```python
from build123d import *

# Parameters (mm, degrees)
COLD_FORMED_SQUARE_HOLLOW_SECTION_GB_T_6_DEPTH = 300


with BuildPart() as part:
    # Sketch1 → Cold-formed square hollow section GB/T 6728-2002 50 X 50 X 4(1) (new body)
    with BuildSketch(Plane.YZ.offset(-88.434077868)):
        with BuildLine():
            Line((-17, -25), (17, -25))
            ThreePointArc((17, -25), (22.656854249, -22.656854249), (25, -17))
            Line((25, -17), (25, 17))
            ThreePointArc((25, 17), (22.656854249, 22.656854249), (17, 25))
            Line((17, 25), (-17, 25))
            ThreePointArc((-17, 25), (-22.656854249, 22.656854249), (-25, 17))
            Line((-25, 17), (-25, -17))
            ThreePointArc((-25, -17), (-22.656854249, -22.656854249), (-17, -25))
        make_face()
        with BuildLine():
            Line((-17, -20), (17, -20))
            ThreePointArc((17, -20), (19.121320344, -19.121320344), (20, -17))
            Line((20, -17), (20, 17))
            ThreePointArc((20, 17), (19.121320344, 19.121320344), (17, 20))
            Line((17, 20), (-17, 20))
            ThreePointArc((-17, 20), (-19.121320344, 19.121320344), (-20, 17))
            Line((-20, 17), (-20, -17))
            ThreePointArc((-20, -17), (-19.121320344, -19.121320344), (-17, -20))
        make_face(mode=Mode.SUBTRACT)
    extrude(amount=COLD_FORMED_SQUARE_HOLLOW_SECTION_GB_T_6_DEPTH)


solid = part.part
```
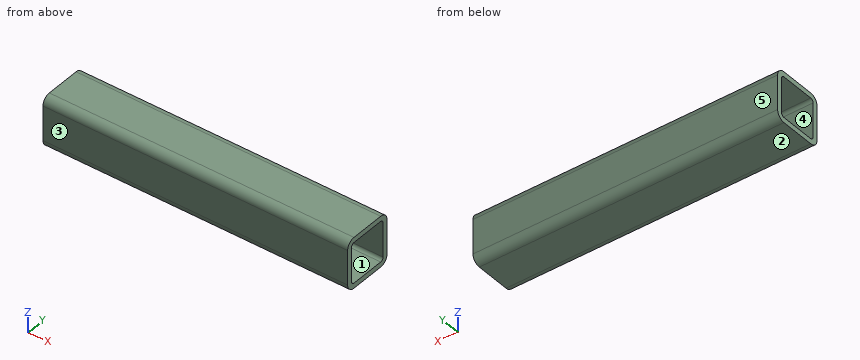
Read the model definition and answer for the solid it produces. Units are mm, in the model's axes. Face numbers are marked on the shaded views. A direction names the side the tool comes from. Coordinates: 2 decimals unless noted, no trailing zeros. Write each loop counter-clockwise with the first axis right and the second up, starting at its lowest first coordinate (ties: lowest second). Pieces come first, ordered by that corner, then holes. Notation, with made-up numbers: (49.5, 89) - (85.5, 89) arc R27 ccw to (85.5, 109) - close; hole circle Ø10 at (10, -11.75). An arc over 180 degrees is marked (long way). Answer as a JSON object with one key per item and string values. Group by question number.
1. A cutting plane is placed at A-A (z = -9). Determine the outline of the cut face in (x, y).
2. Consider L1, parallel to Y at x = 39.5, z = 11; L2, parallel to Y at x = 61, z = 18. Determine where each line is inside the solid, lowest interval first. Write a range as [from, to].
3. A cutting plane is placed at D-D (y = 22.5). Determine the outline of the cut face in (x, z).
4. The mould has two halves that part along Y. Classify the marked faces 1, 2 and 3: +Y half, -Y half, draft (parallel to the pull), parting line (faces both ways), or undercut.
5. Each of these flat-tipped pins is pushed along its axis until it touches: P1, Ø4, axis at x = 171, y = 19.5, coming from the +Z side; P2, Ø4, axis at x = -13.5, y = 20, coming from the +Z side. Where does it stop, or does it pass through?
6. Which of the six approach directions +Z, -Z, +X, -X, +Y, -Y give full straight-line access (tool end or side, diameter ignored) to the marked faces 4 and 5?
7. A cutting plane is placed at C-C (x = 39). Determine the outline of the cut face in (y, z), plus the area to 3 significant figures.
Worked out:
{
 "1": {"outline": "(-88.43, -25) - (211.57, -25) - (211.57, -20) - (-88.43, -20) - close; (-88.43, 20) - (211.57, 20) - (211.57, 25) - (-88.43, 25) - close"},
 "2": {"L1": "y = [-25, -20], [20, 25]", "L2": "y = [-24.94, -19.83], [19.83, 24.94]"},
 "3": {"outline": "(-88.43, -22.81) - (211.57, -22.81) - (211.57, 22.81) - (-88.43, 22.81) - close"},
 "4": {"face 1": "undercut", "face 2": "draft", "face 3": "-Y half"},
 "5": {"P1": "stops at z = 24.98", "P2": "stops at z = 24.94"},
 "6": {"face 4": "+X, -X", "face 5": "+Z, -Z, +X, -X, +Y"},
 "7": {"outline": "(-25, -17) arc R8 ccw to (-17, -25) - (17, -25) arc R8 ccw to (25, -17) - (25, 17) arc R8 ccw to (17, 25) - (-17, 25) arc R8 ccw to (-25, 17) - close; hole (-20, -17) arc R3 ccw to (-17, -20) - (17, -20) arc R3 ccw to (20, -17) - (20, 17) arc R3 ccw to (17, 20) - (-17, 20) arc R3 ccw to (-20, 17) - close", "area": "853 mm²"}
}
